```python
from build123d import *

# Parameters (mm, degrees)
SKETCH_1_R               = 5
EXTRUDE_1_DEPTH          = 62.5
CHAMFER_1_SIZE           = 0.5
SKETCH_2_W               = 4.472118267
SKETCH_2_H               = 12.857340018
CUT_EXTRUDE_1_DEPTH      = 55.5
PATTERN_CIRCULAR_1_COUNT = 3
HOLE_WIZARD_M4_1_D       = 3.3
HOLE_WIZARD_M4_1_DEPTH   = 15.5
HOLE_WIZARD_M4_1_TIP     = 0.991420021


with BuildPart() as part:
    # 草图1 → 凸台-拉伸1 (new body)
    with BuildSketch(Plane(origin=(0, 0, 0), x_dir=(0, 0, -1), z_dir=(1, 0, 0))):
        Circle(SKETCH_1_R)
    extrude(amount=EXTRUDE_1_DEPTH)

    # 倒角1
    chamfer_1_edges = [part.edges().sort_by_distance(p)[0] for p in [
        (0, 0, 5),
        (62.5, 0, 5),
    ]]
    chamfer(chamfer_1_edges, length=CHAMFER_1_SIZE)

    # 草图2 → 切除-拉伸1 (cut)
    with BuildSketch(Plane(origin=(62.5, 0, 0), x_dir=(0, 0, -1), z_dir=(1, 0, 0))):
        with Locations((-6.536059134, -0.104972075)):
            Rectangle(SKETCH_2_W, SKETCH_2_H)
    cut_extrude_1 = extrude(amount=-CUT_EXTRUDE_1_DEPTH, mode=Mode.SUBTRACT)

    # 阵列(圆周)1: 切除-拉伸1 ×3 about axis
    pattern_circular_1_axis = Axis((0, 0, 0), (1, 0, 0))
    for i in range(1, PATTERN_CIRCULAR_1_COUNT):
        add(cut_extrude_1.rotate(pattern_circular_1_axis, i * 360 / PATTERN_CIRCULAR_1_COUNT), mode=Mode.SUBTRACT)

    # M4 螺纹孔1
    with Locations(Plane.ZY):
        with Locations((0, 0)):
            Hole(HOLE_WIZARD_M4_1_D / 2, depth=HOLE_WIZARD_M4_1_DEPTH)
            with Locations((0, 0, -(HOLE_WIZARD_M4_1_DEPTH + HOLE_WIZARD_M4_1_TIP / 2))):  # 118° drill point
                Cone(0, HOLE_WIZARD_M4_1_D / 2, HOLE_WIZARD_M4_1_TIP, mode=Mode.SUBTRACT)


solid = part.part
```
Geometry: final body of the model. Coordinates: model frame, mm. A direction names the side the tool comes from. Round coordinates to 2 decimals unless told otherwise and drop trailing zeros. Order: outer loops, then holes, each group sorted by start corner. A loop starts at its lowest first (then second) coordinate and runs counter-clockwise, first axis right, second up. Notation, with made-up numbers: (-32, 4.5) - (-22, 4.5) arc R20 ccw to (-22, 17.5) - close; hole circle Ø9 at (-2.75, 50). An arc over 180 degrees is marked (long way). Write item = value, one per line. Start each with the question number.
Q1. Pull-direction query (Y, two-part tool) for faces 6 (the flat face through (35.138, -3.706, -2.181)), 7 (the cylindrical face through (7.858, 1.115, 1.216)), 8 (the flat face through (62.5, 0, 0)); classes: +Y half, -Y half, draft (parallel to the pull), parting line (faces both ways), or undercut.
Q2. Access query for faces 1 (the conical face through (16.3, -0.3, -0.1)), 2 (the flat face through (35, 0, 4.3)), 3 (the flat face through (0, -2, 0)), 4 (the flat face through (7, 4, -2)), 5 (the flat face through (7, -4, -2)). Directions: +Z, -Z, +X, -X, +Y, -Y. A direction counts if a zero-diameter tool reaches every point of the face in a straight line with its end or side. Return the directions, or none.
Q3. Cut plane B-B on x = 39.5. Return the cut outline in (y, z).
Q4. Pin query (flat end, axial travel): pin 1 (6 mm diameter, centred on x = 15, y = -2, fed in from +Z); pin 2 (6 mm diameter, centred on y = 4, z = -3, fed in from +X); pin 3 (1 mm diameter, centred on x = 11.5, z = -1, fed in from -Y); pin 4 (1.5 mm diameter, centred on x = 39.5, z = -2, fed in from +Y). Return the tip coordinate at first contact, or that it passes through.
Q5. Cut plane A-A on x = 13.5. Return the cut outline in (y, z), and give its area (3 significant figures).
Q6. Ray query, line 1 (Z direction, x = 11, y = 0); line 2 (Y direction, x = 3.75, z = 0); line 3 (Z direction, x = 8.5, y = 0.75). Return the intervals inside material, ascending. Write a range as from..to.
Outcome:
q1.face_6 = -Y half
q1.face_7 = undercut
q1.face_8 = draft
q2.face_1 = -X
q2.face_2 = +Z, +X, +Y, -Y
q2.face_3 = +Z, -Z, -X, +Y, -Y
q2.face_4 = -Z, +X, +Y
q2.face_5 = -Z, +X, -Y
q3.outline = (-5, 0.06) - (-2.45, -4.36) arc R5 ccw to (2.45, -4.36) - (5, 0.06) arc R5 ccw to (2.55, 4.3) - (-2.55, 4.3) arc R5 ccw to start
q4.pin_1 = 4.3
q4.pin_2 = 62.5
q4.pin_3 = -4.68
q4.pin_4 = 4.24
q5.outline = (-5, 0.06) - (-2.45, -4.36) arc R5 ccw to (2.45, -4.36) - (5, 0.06) arc R5 ccw to (2.55, 4.3) - (-2.55, 4.3) arc R5 ccw to start; hole circle Ø3.3 at (0, 0)
q5.area = 62.7 mm^2
q6.line_1 = -5..-1.65, 1.65..4.3
q6.line_2 = -5..-1.65, 1.65..5
q6.line_3 = -4.94..-1.47, 1.47..4.3
